Source: three-view drawing plus pictorial views. Frame: mm from the lowest corner of the part. Give positions to 0.01 mm unless a question says otherwise; leave off trailing zeros. Loops run counter-clockwise (first coordinate to the right, second up) from the corner with the lowest first, then second, coordinate; pieces in that order, holes last. Notation, with made-up numbers: (69, 5) -> (109, 5) arc R21 ccw to (109, 37) -> close; hole circle Ø6 at (18.5, 49.5). An arc over 180 degrees is marked (long way). Answer in a Markdown table with one row per item. Add a question column.
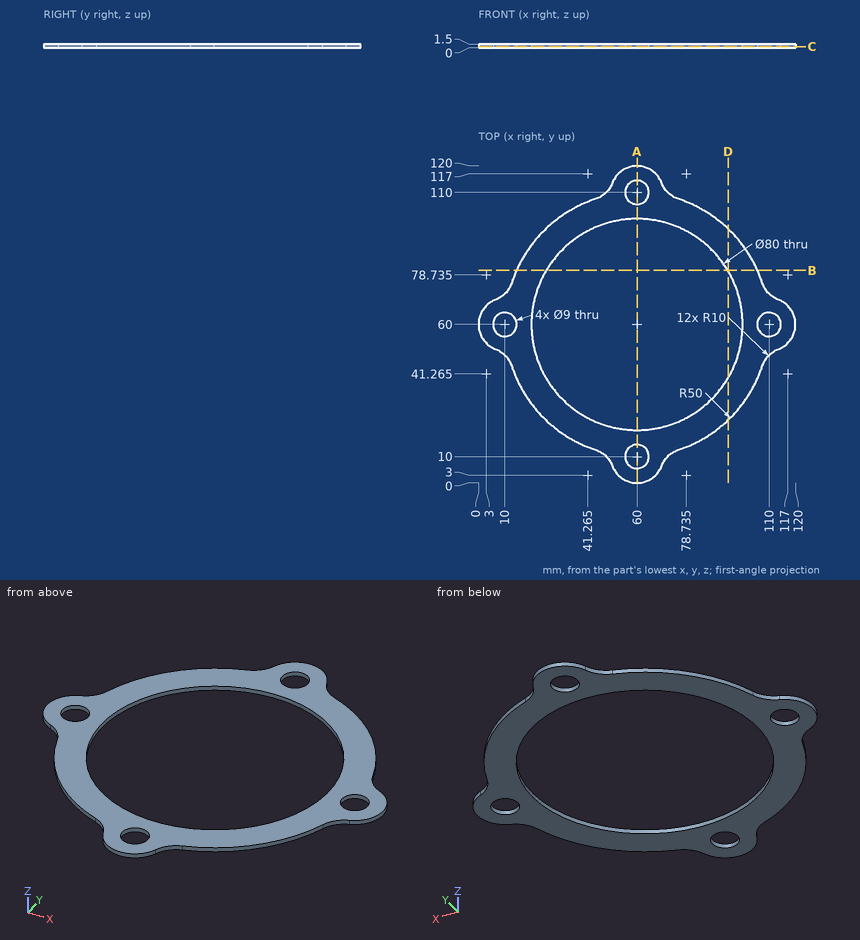
(1) Cut plane C-C on z = 0.55. Return the cut outline in (x, y) (1 decimal).
(2) Cut plane D-D on x = 94.5. Return the cut outline in (y, z), then the cut area to 3 significant figures.
(3) Material intervals for line 1 along Y through (x, z) = (60, 0.5); line 2 along Y through (x, z) = (10, 0.6); line 3 along Y through (x, z) = (82.5, 0.1), sorted ascending. Write a range as from..to.
(4) Cut plane B-B on y = 80.5. Return the cut outline in (x, z), then the cut area to 3 significant figures.
(5) Pin query (flat end, axial travel): pin 1 Ø7 at (x, y) = (60, 110) entering from +Z. Return the tip coordinate at first contact, or that it passes through.
(6) Cut plane A-A on x = 60. Return the cut outline in (y, z), then the cut area to 3 significant figures.
Answer list:
| question | item | result |
|---|---|---|
| 1 | outline | (6.5, 50.6) arc R10 cw to (12.5, 44.4) arc R50 ccw to (44.4, 12.5) arc R10 cw to (50.6, 6.5) arc R10 ccw to (69.4, 6.5) arc R10 cw to (75.6, 12.5) arc R50 ccw to (107.5, 44.4) arc R10 cw to (113.5, 50.6) arc R10 ccw to (113.5, 69.4) arc R10 cw to (107.5, 75.6) arc R50 ccw to (75.6, 107.5) arc R10 cw to (69.4, 113.5) arc R10 ccw to (50.6, 113.5) arc R10 cw to (44.4, 107.5) arc R50 ccw to (12.5, 75.6) arc R10 cw to (6.5, 69.4) arc R10 ccw to start; hole circle Ø9 at (10, 60); hole circle Ø80 at (60, 60); hole circle Ø9 at (60, 10); hole circle Ø9 at (60, 110); hole circle Ø9 at (110, 60) |
| 2 | outline | (23.81, 0) -> (39.76, 0) -> (39.76, 1.5) -> (23.81, 1.5) -> close; (80.24, 0) -> (96.19, 0) -> (96.19, 1.5) -> (80.24, 1.5) -> close |
| 2 | area | 47.8 mm² |
| 3 | line 1 | y = 0..5.5, 14.5..20, 100..105.5, 114.5..120 |
| 3 | line 2 | y = 48.41..55.5, 64.5..71.59 |
| 3 | line 3 | y = 15.35..26.93, 93.07..104.65 |
| 4 | outline | (14.4, 0) -> (25.65, 0) -> (25.65, 1.5) -> (14.4, 1.5) -> close; (94.35, 0) -> (105.6, 0) -> (105.6, 1.5) -> (94.35, 1.5) -> close |
| 4 | area | 33.8 mm² |
| 5 | pin 1 | passes through |
| 6 | outline | (0, 0) -> (5.5, 0) -> (5.5, 1.5) -> (0, 1.5) -> close; (14.5, 0) -> (20, 0) -> (20, 1.5) -> (14.5, 1.5) -> close; (100, 0) -> (105.5, 0) -> (105.5, 1.5) -> (100, 1.5) -> close; (114.5, 0) -> (120, 0) -> (120, 1.5) -> (114.5, 1.5) -> close |
| 6 | area | 33.0 mm² |
